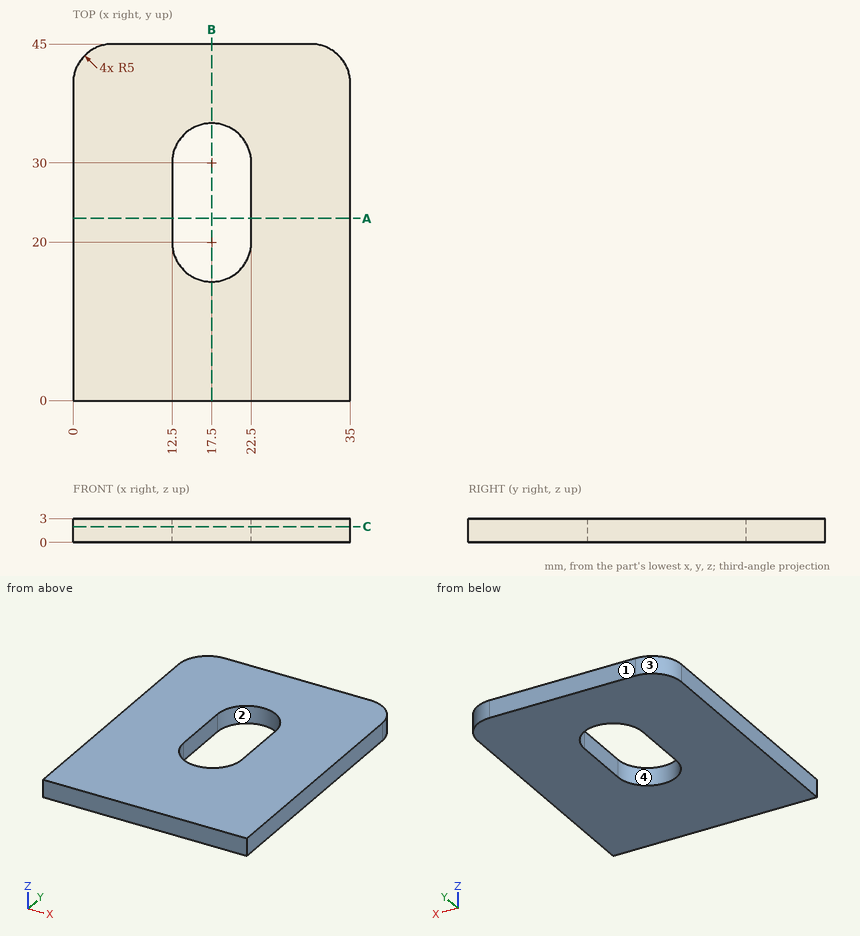
The drawing under review shows one solid part. Ordinate dimensions are in mm from its lowest x, y, z. Round coordinates to 2 decimals unless told otherwise and drop trailing zeros. Loops run counter-clockwise (first coordinate to the right, second up) from the corner with the lowest first, then second, coordinate; pieces in that order, holes last. Notation, with made-up numbers: (-33, -3) -> (-9, -3) arc R23 ccw to (-9, 33) -> close; hole circle Ø7 at (3.5, 39.25). An arc over 180 degrees is marked (long way). Answer in a Markdown table with one row per item.
1) Wall thickness on line 1 along X through (y, z) = (22, 0.55); line 2 along Y through (x, z) = (18, 2.7); line 3 along Y through (x, z) = (14, 0.2): over which ranges is each line inside the solid? List them lowest first.
Taken from the geometry:
| item | result |
|---|---|
| line 1 | x = 0 to 12.5, 22.5 to 35 |
| line 2 | y = 0 to 15.03, 34.97 to 45 |
| line 3 | y = 0 to 16.43, 33.57 to 45 |
2) Consider section B-B, the plane x = 17.5. Write out the cut boundary in (y, z), plus the area to 3 significant figures.
Taken from the geometry:
| item | result |
|---|---|
| outline | (0, 0) -> (15, 0) -> (15, 3) -> (0, 3) -> close; (35, 0) -> (45, 0) -> (45, 3) -> (35, 3) -> close |
| area | 75.0 mm² |
3) Consider section C-C, the plane z = 2. Write out the cut boundary in (x, y), plus the area to 3 significant figures.
Taken from the geometry:
| item | result |
|---|---|
| outline | (0, 0) -> (35, 0) -> (35, 40) arc R5 ccw to (30, 45) -> (5, 45) arc R5 ccw to (0, 40) -> close; hole (12.5, 20) arc R5 ccw to (22.5, 20) -> (22.5, 30) arc R5 ccw to (12.5, 30) -> close |
| area | 1,390 mm² |
4) Draft analysis for pull direction X (two halves, no side actions). For the marked faces 1, 2, 3 and 4, state which applies: pulls with the +X half, pulls with the -X half, needs draft (parallel to the pull), parting line crosses it, or undercut.
Taken from the geometry:
| item | result |
|---|---|
| face 1 | needs draft |
| face 2 | undercut |
| face 3 | pulls with the -X half |
| face 4 | undercut |
5) Consider section A-A, the plane y = 23. Write out the cut boundary in (x, z).
Taken from the geometry:
| item | result |
|---|---|
| outline | (0, 0) -> (12.5, 0) -> (12.5, 3) -> (0, 3) -> close; (22.5, 0) -> (35, 0) -> (35, 3) -> (22.5, 3) -> close |
